Could you check a few things on this drawing? It's one solid part, dimensions in mm from its lowest x, y, z. A direction names the side the tool comes from. Give positions to 0.01 mm unless a question says otherwise; leave off trailing zeros. Loops run counter-clockwise (first coordinate to the right, second up) from the corner with the lowest first, then second, coordinate; pieces in that order, holes last.
1. For P1, Ø1.8, axis at y = 70, z = 61, coming from the -X side; P2, Ø4, axis at x = 17.5, z = 48.5, coming from the +Y side; P3, Ø4, axis at x = 12, z = 7, coming from the +Y side; P4, Ø12, axis at y = 62.5, z = 45.5, coming from the +X side, each with a flat end and sliding along its axis, tell me the tip position at first contact or that it passes through.
2. Imagine slicing it at D-D (x = 72.5). List the corners of the cut face in (y, z) for me, plus the area to 3 significant figures.
3. Imagine slicing it at A-A (z = 23). List the corners of the cut face in (x, y) for me.
4. Imagine slicing it at C-C (y = 73). List the corners of the cut face in (x, z) for me.
5. For the marked faces 1 and 2, which set-ups out of +Z, -Z, +X, -X, +Y, -Y let a thin tool reach every point of the face, with its end or its side?
6. I need wall thicknesses on line 1 along Y through (x, z) = (80, 10); line 2 along Z through (x, y) = (5.5, 30.5); line 3 along Y through (x, z) = (29.5, 49). Which ranges of each line are inside material? Lowest first, please.
7. Imagine slicing it at B-B (x = 50). List the corners of the cut face in (y, z) for me.
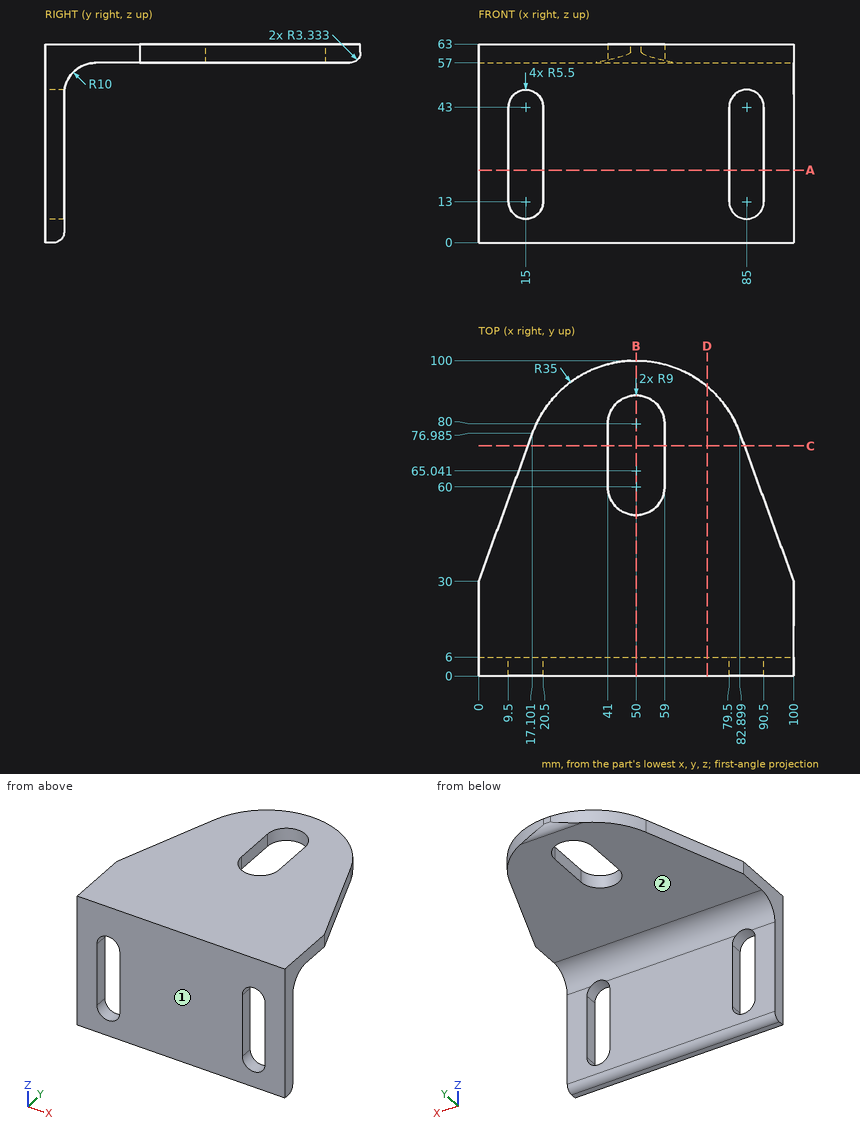
Derived:
1. P1: stops at x = 14.23
1. P2: stops at y = 6.63
1. P3: stops at y = 6
1. P4: passes through
2. outline: (0, 0) - (2.67, 0) arc R3.33 ccw to (6, 3.33) - (6, 47) arc R10 cw to (16, 57) - (91.85, 57) - (91.85, 63) - (0, 63) - close
2. area: 912 mm2
3. outline: (0, 0) - (9.5, 0) - (9.5, 6) - (0, 6) - close; (20.5, 0) - (79.5, 0) - (79.5, 6) - (20.5, 6) - close; (90.5, 0) - (100, 0) - (100, 6) - (90.5, 6) - close
4. outline: (15.65, 57) - (41, 57) - (41, 63) - (15.65, 63) - close; (59, 57) - (84.35, 57) - (84.35, 63) - (59, 63) - close
5. face 1: +Z, -Z, +X, -X, -Y
5. face 2: -Z, +X, -X, +Y
6. line 1: y = 0 to 6
6. line 2: z = 57 to 63
6. line 3: y = 0 to 6.2
7. outline: (0, 0) - (2.67, 0) arc R3.33 ccw to (6, 3.33) - (6, 47) arc R10 cw to (16, 57) - (51, 57) - (51, 63) - (0, 63) - close; (89, 57) - (96.67, 57) arc R3.33 ccw to (100, 60.33) - (100, 63) - (89, 63) - close
